For this review, use the dimensioned drawing (mm, ordinates from the lowest corner) and the shaded views. A direction names the side the tool comes from. Give positions to 0.01 mm unless a question says otherwise; leave off trailing zeros. Order: outer loops, then holes, each group sorted by start corner. A loop starts at its lowest first (then second) coordinate and runs counter-clockwise, first axis right, second up.
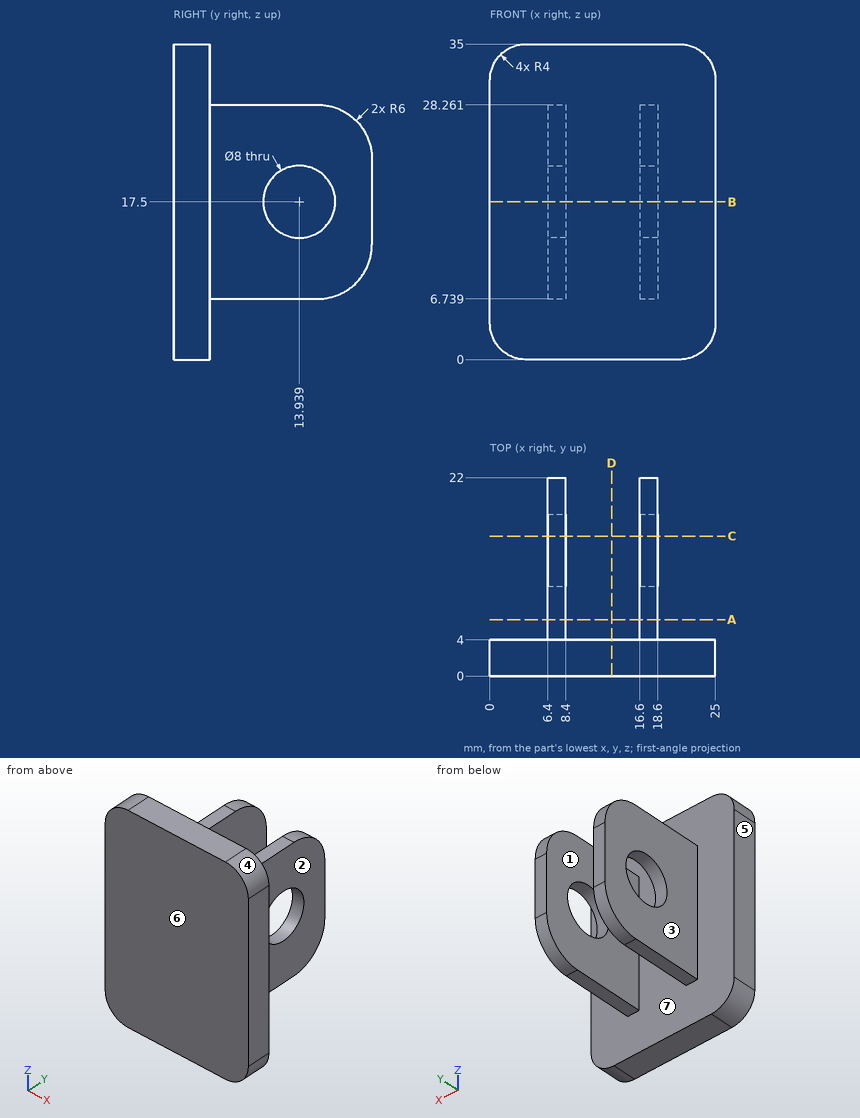
1. Take a section at B-B (z = 17.5). State the section outline as (x, y) points, then the cut area to 3 significant figures.
Recorded:
outline: (0, 0) - (25, 0) - (25, 4) - (18.6, 4) - (18.6, 9.94) - (16.6, 9.94) - (16.6, 4) - (8.4, 4) - (8.4, 9.94) - (6.4, 9.94) - (6.4, 4) - (0, 4) - close; (6.4, 17.94) - (8.4, 17.94) - (8.4, 22) - (6.4, 22) - close; (16.6, 17.94) - (18.6, 17.94) - (18.6, 22) - (16.6, 22) - close
area: 140 mm2
2. Draft analysis for pull direction X (two halves, no side actions). For the marked faces 5, 6 and 7, state which applies: pulls with the +X half, pulls with the -X half, needs draft (parallel to the pull), parting line crosses it, or undercut.
Recorded:
face 5: pulls with the -X half
face 6: needs draft
face 7: undercut
3. Take a section at C-C (y = 15.5). State the section outline as (x, z) points.
Recorded:
outline: (6.4, 6.74) - (8.4, 6.74) - (8.4, 13.82) - (6.4, 13.82) - close; (6.4, 21.18) - (8.4, 21.18) - (8.4, 28.26) - (6.4, 28.26) - close; (16.6, 6.74) - (18.6, 6.74) - (18.6, 13.82) - (16.6, 13.82) - close; (16.6, 21.18) - (18.6, 21.18) - (18.6, 28.26) - (16.6, 28.26) - close
4. Take a section at D-D (x = 13.5). State the section outline as (y, z) points.
Recorded:
outline: (0, 0) - (4, 0) - (4, 35) - (0, 35) - close
5. Machinability: for the marked faces 1, 2, 3 and 4, which of the approach directions +Z, -Z, +X, -X, +Y, -Y give a long, thin tool a straight path to every point of the face, cutting with its end or side? Answer none if there is none.
Recorded:
face 1: +Z, -Z, +Y
face 2: +Z, -Z, +X, +Y
face 3: +Z, -Z, -X, +Y
face 4: +Z, +X, +Y, -Y
6. For pin 1 (6 mm diameter, centred on y = 16, z = 22, fed in from -X); pin 2 (1 mm diameter, centred on x = 17.5, y = 11, fed in from +Z); pin 3 (2 mm diameter, centred on x = 7.5, y = 7.5, fed in from -Z); pin 4 (5 mm diameter, centred on y = 13.94, z = 17.5, fed in from +X), all flat-tipped, find the tip position at first contact; note any pin that passes through.
Recorded:
pin 1: stops at x = 6.4
pin 2: stops at z = 28.26
pin 3: stops at z = 6.74
pin 4: passes through
7. Take a section at A-A (y = 6.25). State the section outline as (x, z) points.
Recorded:
outline: (6.4, 6.74) - (8.4, 6.74) - (8.4, 28.26) - (6.4, 28.26) - close; (16.6, 6.74) - (18.6, 6.74) - (18.6, 28.26) - (16.6, 28.26) - close
8. For line 1 along X through (y, z) = (13.25, 13); line 2 along Y through (x, z) = (17.3, 17.5); line 3 along Y through (x, z) = (6, 7), list the stretches that pass through material, from the lowest coordinate up.
Recorded:
line 1: x = 6.4 to 8.4, 16.6 to 18.6
line 2: y = 0 to 9.94, 17.94 to 22
line 3: y = 0 to 4
